from build123d import *

# Parameters (mm, degrees)
SKETCH_1_W                   = 12
SKETCH_1_H                   = 45
EXTRUDE_1_DEPTH              = 5
HOLE_WIZARD_M6_1_D           = 5
HOLE_WIZARD_M6_1_CSINK_D     = 6.05
HOLE_WIZARD_M6_1_CSINK_ANGLE = 90
CUT_EXTRUDE_1_REACH          = 27.986
SKETCH_3_R                   = 3.25
CHAMFER_1_SIZE               = 2


with BuildPart() as part:
    # 草图1 → 凸台-拉伸1 (new, symmetric)
    with BuildSketch(Plane.XY):
        Rectangle(SKETCH_1_W, SKETCH_1_H)
    extrude(amount=EXTRUDE_1_DEPTH, both=True)

    # M6 螺纹孔1 (through all)
    with Locations(Plane(origin=(0, -16, 5), x_dir=(1, 0, 0), z_dir=(0, 0, 1))):
        with Locations((0, 0)):
            hole_wizard_m6_1 = CounterSinkHole(HOLE_WIZARD_M6_1_D / 2, HOLE_WIZARD_M6_1_CSINK_D / 2, counter_sink_angle=HOLE_WIZARD_M6_1_CSINK_ANGLE)

    # 草图3 → 切除-拉伸1 (cut, up to next)
    with BuildSketch(Plane.ZY.offset(6), mode=Mode.PRIVATE) as cut_extrude_1_sk1:
        with Locations((0, 7.5)):
            Circle(SKETCH_3_R)
    cut_extrude_1_tool1 = extrude(cut_extrude_1_sk1.sketch, amount=-CUT_EXTRUDE_1_REACH, mode=Mode.PRIVATE) & part.part
    # 草图3 → 切除-拉伸1 (cut, up to next)
    with BuildSketch(Plane.ZY.offset(6), mode=Mode.PRIVATE) as cut_extrude_1_sk2:
        with Locations((0, -7.5)):
            Circle(SKETCH_3_R)
    cut_extrude_1_tool2 = extrude(cut_extrude_1_sk2.sketch, amount=-CUT_EXTRUDE_1_REACH, mode=Mode.PRIVATE) & part.part
    add(cut_extrude_1_tool1.solids().sort_by_distance((-6, 7.5, 0))[0], mode=Mode.SUBTRACT)
    add(cut_extrude_1_tool2.solids().sort_by_distance((-6, -7.5, 0))[0], mode=Mode.SUBTRACT)

    # 镜向1: M6 螺纹孔1 across plane
    add(hole_wizard_m6_1.mirror(Plane.ZX), mode=Mode.SUBTRACT)

    # 倒角1
    chamfer_1_edges = [part.edges().sort_by_distance(p)[0] for p in [
        (6, -22.5, 0),
        (-6, -22.5, 0),
        (-6, 22.5, 0),
        (6, 22.5, 0),
    ]]
    chamfer(chamfer_1_edges, length=CHAMFER_1_SIZE)


solid = part.part
Here's how the part is built. I have some questions about the finished solid (model axes, mm). Coordinates: 2 decimals unless noted, no trailing zeros. Order: outer loops, then holes, each group sorted by start corner. A loop starts at its lowest first (then second) coordinate and runs counter-clockwise, first axis right, second up. Notation, with made-up numbers: (-10.75, -15) -> (29.25, -15) arc R23 cw to (29.25, 17) -> close; hole circle Ø3 at (-6, 1). An arc over 180 degrees is marked (long way). Answer in a Markdown table with one row per item.
(1) I want a section at B-B on y = 7.5. List the corners of the cut face in (x, z) for me.
Answer key:
| item | result |
|---|---|
| outline | (-6, -5) -> (6, -5) -> (6, -3.25) -> (-6, -3.25) -> close; (-6, 3.25) -> (6, 3.25) -> (6, 5) -> (-6, 5) -> close |
(2) Thinking about a two-plate mould opening in Z: for faces 1 (the face through (0, 22.5, 0)), 2 (the face through (-0.084, -4.278, -0.423)), 3 (the face through (0, 0, 5)), which applies, +Z half, -Z half, draft (parallel to the pull), parting line (faces both ways), or undercut?
Answer key:
| item | result |
|---|---|
| face 1 | draft |
| face 2 | undercut |
| face 3 | +Z half |
(3) I want a section at C-C on x = 0. List the corners of the cut face in (y, z) for me (3 decimals).
Answer key:
| item | result |
|---|---|
| outline | (-22.5, -5) -> (-18.5, -5) -> (-18.5, 4.475) -> (-19.025, 5) -> (-22.5, 5) -> close; (-13.5, -5) -> (13.5, -5) -> (13.5, 4.475) -> (12.975, 5) -> (-12.975, 5) -> (-13.5, 4.475) -> close; (18.5, -5) -> (22.5, -5) -> (22.5, 5) -> (19.025, 5) -> (18.5, 4.475) -> close; hole circle Ø6.5 at (-7.5, 0); hole circle Ø6.5 at (7.5, 0) |
(4) I want a section at A-A on z = 0. List the corners of the cut face in (x, y) for me.
Answer key:
| item | result |
|---|---|
| outline | (-6, -20.5) -> (-4, -22.5) -> (4, -22.5) -> (6, -20.5) -> (6, -10.75) -> (-6, -10.75) -> close; (-6, -4.25) -> (6, -4.25) -> (6, 4.25) -> (-6, 4.25) -> close; (-6, 10.75) -> (6, 10.75) -> (6, 20.5) -> (4, 22.5) -> (-4, 22.5) -> (-6, 20.5) -> close; hole circle Ø5 at (0, -16); hole circle Ø5 at (0, 16) |
(5) Please list where these lines run through material, in increasing order: probe 1 along Y at (x, z) = (0, 0); probe 2 along Y at (x, z) = (-5, -1); probe 3 along Y at (x, z) = (4.25, -2.75).
Answer key:
| item | result |
|---|---|
| probe 1 | -22.5 to -18.5, -13.5 to -10.75, -4.25 to 4.25, 10.75 to 13.5, 18.5 to 22.5 |
| probe 2 | -21.5 to -10.59, -4.41 to 4.41, 10.59 to 21.5 |
| probe 3 | -22.25 to -9.23, -5.77 to 5.77, 9.23 to 22.25 |
(6) I want a section at D-D on x = -4.75. List the corners of the cut face in (y, z) for me.
Answer key:
| item | result |
|---|---|
| outline | (-21.75, -5) -> (21.75, -5) -> (21.75, 5) -> (-21.75, 5) -> close; hole circle Ø6.5 at (-7.5, 0); hole circle Ø6.5 at (7.5, 0) |
